For this review, take the finished solid that the model builds, in its own axes (mm). Face numbers are marked on the shaded views. A direction names the side the tool comes from. Give positions to 0.01 mm unless a question says otherwise; leave off trailing zeros. Write each loop counter-clockwise with the first axis right and the second up, starting at its lowest first coordinate (ties: lowest second). Pieces come first, ordered by that corner, then holes. Notation, with made-up numbers: (24.25, 34) -> (61.25, 34) arc R15 cw to (61.25, 49) -> close; hole circle Ø5 at (33.5, -7). An arc over 180 degrees is marked (long way). Answer as CSV lines item,"result".
```python
from build123d import *

# Parameters (mm, degrees)
EDGE_CHAMFER_2X45_SIZE = 2


with BuildPart() as part:
    # Shaft Profile Sketch → Stepped Shaft Revolve (revolve)
    with BuildSketch(Plane.XY):
        Polygon((-58.5, 0), (-58.5, -5), (-46.5, -5), (-46.5, -8), (-26.5, -8), (-26.5, -12.5), (-16.5, -12.5), (-16.5, -10), (11.5, -10), (11.5, -7.5), (36.5, -7.5), (36.5, -5.5), (58.5, -5.5), (58.5, 0), align=None)
    revolve(axis=Axis((-58.5, 0, 0), (1, 0, 0)))

    # Edge Chamfer 2x45°
    edge_chamfer_2x45_edges = [part.edges().sort_by_distance(p)[0] for p in [
        (58.5, 5.5, 0),
        (-58.5, 5, 0),
    ]]
    chamfer(edge_chamfer_2x45_edges, length=EDGE_CHAMFER_2X45_SIZE)


solid = part.part
```
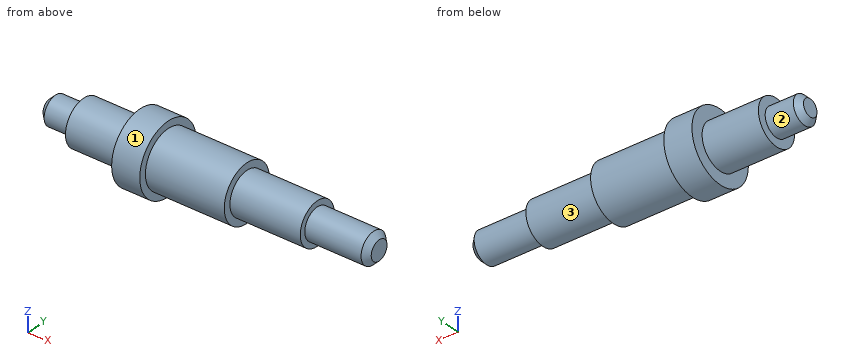
Q1. Add section C-C (x = -45.5). Write out the cut boundary in (y, z).
Answer block:
outline,"circle Ø16 at (0, 0)"
Q2. Clearance check with flat-ended pins moving along their axes: pin 1 (3 mm diameter, centred on x = -8.5, y = -4.5, fed in from -Z); pin 2 (10 mm diameter, centred on y = -4.5, z = 3, fed in from +X); pin 3 (1.5 mm diameter, centred on x = 44, z = 1.5, fed in from -Y); pin 4 (2 mm diameter, centred on x = -7.5, y = -9, fed in from -Z). State where each tip first meets the part, or that it passes through.
Answer block:
pin 1,"stops at z = -9.54"
pin 2,"stops at x = 58.5"
pin 3,"stops at y = -5.45"
pin 4,"stops at z = -6"
Q3. Add section A-A (z = 0). Write out the cut boundary in (x, y).
Answer block:
outline,"(-58.5, -3) -> (-56.5, -5) -> (-46.5, -5) -> (-46.5, -8) -> (-26.5, -8) -> (-26.5, -12.5) -> (-16.5, -12.5) -> (-16.5, -10) -> (11.5, -10) -> (11.5, -7.5) -> (36.5, -7.5) -> (36.5, -5.5) -> (56.5, -5.5) -> (58.5, -3.5) -> (58.5, 3.5) -> (56.5, 5.5) -> (36.5, 5.5) -> (36.5, 7.5) -> (11.5, 7.5) -> (11.5, 10) -> (-16.5, 10) -> (-16.5, 12.5) -> (-26.5, 12.5) -> (-26.5, 8) -> (-46.5, 8) -> (-46.5, 5) -> (-56.5, 5) -> (-58.5, 3) -> close"
Q4. Add section D-D (z = -6.5). Write out the cut boundary in (x, y).
Answer block:
outline,"(-46.5, -4.66) -> (-26.5, -4.66) -> (-26.5, -10.68) -> (-16.5, -10.68) -> (-16.5, -7.6) -> (11.5, -7.6) -> (11.5, -3.74) -> (36.5, -3.74) -> (36.5, 3.74) -> (11.5, 3.74) -> (11.5, 7.6) -> (-16.5, 7.6) -> (-16.5, 10.68) -> (-26.5, 10.68) -> (-26.5, 4.66) -> (-46.5, 4.66) -> close"
Q5. To check wall thickness, follow probe 1 along X at (y, z) = (10, -6.25); probe 2 along X at (y, z) = (-9, -0.25); probe 3 along Z at (x, y) = (-33.5, 0.5). State the ranges of each line that lie inside material, in increasing order. Write a range as [from, to].
Answer block:
probe 1,"x = [-26.5, -16.5]"
probe 2,"x = [-26.5, 11.5]"
probe 3,"z = [-7.98, 7.98]"
Q6. For the marked faces 1, 2 and 3, list the 3-axis set-ups (+Z, -Z, +X, -X, +Y, -Y) from which the entire face can be reached by the end or side of a thin tool; tool diameter is ignored.
Answer block:
face 1,"+X, -X"
face 2,"-X"
face 3,"+X"
